Read the model definition and answer for the solid it produces. Units are mm, in the model's axes. A direction names the side the tool comes from. Round coordinates to 2 decimals unless told otherwise and drop trailing zeros. Loops run counter-clockwise (first coordinate to the right, second up) from the corner with the lowest first, then second, coordinate; pieces in that order, holes last. Notation, with made-up numbers: (23.5, 23.5) - (42.5, 23.5) arc R27 ccw to (42.5, 44.5) - close; hole circle Ø9 at (36.5, -9). An arc over 180 degrees is marked (long way). Use one line per item in the form item = value. Start each with the question number.
```python
from build123d import *

# Parameters (mm, degrees)
SKETCH1_R           = 45
SKETCH1_R_2         = 25
BOSS_EXTRUDE1_DEPTH = 15
CUT_EXTRUDE1_START  = -3
SKETCH2_R           = 45
SKETCH2_R_2         = 40
CUT_EXTRUDE1_DEPTH  = 3
SKETCH3_R           = 2
CUT_EXTRUDE2_DEPTH  = 11
CHAMFER1_SIZE       = 1


with BuildPart() as part:
    # Sketch1 → Boss-Extrude1 (new body)
    with BuildSketch(Plane.XY):
        Circle(SKETCH1_R)
        Circle(SKETCH1_R_2, mode=Mode.SUBTRACT)
    extrude(amount=BOSS_EXTRUDE1_DEPTH)

    # Sketch2 → Cut-Extrude1 (cut)
    with BuildSketch(Plane.XY.offset(15).offset(CUT_EXTRUDE1_START)):
        Circle(SKETCH2_R)
        Circle(SKETCH2_R_2, mode=Mode.SUBTRACT)
    extrude(amount=CUT_EXTRUDE1_DEPTH, mode=Mode.SUBTRACT)

    # Sketch3 → Cut-Extrude2 (cut)
    with BuildSketch(Plane(origin=(0, 0, 0), x_dir=(-1, 0, 0), z_dir=(0, 0, -1))):
        with Locations((0, 36.5)):
            Circle(SKETCH3_R)
        with Locations((31.609927238, 18.25)):
            Circle(SKETCH3_R)
        with Locations((31.609927238, -18.25)):
            Circle(SKETCH3_R)
        with Locations((0, -36.5)):
            Circle(SKETCH3_R)
        with Locations((-31.609927238, -18.25)):
            Circle(SKETCH3_R)
        with Locations((-31.609927238, 18.25)):
            Circle(SKETCH3_R)
    extrude(amount=-CUT_EXTRUDE2_DEPTH, mode=Mode.SUBTRACT)

    # Chamfer1
    chamfer1_edges = [part.edges().sort_by_distance(p)[0] for p in [
        (-40, 0, 15),
        (-25, 0, 0),
    ]]
    chamfer(chamfer1_edges, length=CHAMFER1_SIZE)


solid = part.part
```
1) A cutting plane is placed at B-B on z = 6.75. Write down the section's boundary in (x, y), plus the area to 3 significant figures.
2) For faces 5 (the flat face through (-0.5, -25.5, 15)), 6 (the flat face through (32, -18, 11)), 7 (the cylindrical face through (-8.67, -39.05, 12.99)), determine the directions among +Z, -Z, +X, -X, +Y, -Y from which every point of the face is accessible in a straight line to the end or side of a thin tool.
3) A cutting plane is placed at A-A on y = 0. Write down the section's boundary in (x, z).
4) Determine the mould class of faces 1 (the flat face through (-30.2, -26.5, 12)), 2 (the flat face through (-32, 18, 11)), 3 (the cylindrical face through (30.535, -16.564, 5.423)), 4 (the cylindrical face through (20.765, -39.923, 5.916)) for opening direction X: +X half, -X half, draft (parallel to the pull), parting line (faces both ways), or undercut.
5) Straight lines are drawn through the part: line 1 (Y direction, x = 0, z = 8.75); line 2 (X direction, y = -0.5, z = 10.25) (3 decimals); line 3 (Y direction, x = 7.5, z = 11). For each, find the intervals that lie inside material, in ascending order. Write a range as from..to.
6) Flat-ended cylindrical pins translate along their axes: pin 1 (3 mm diameter, centred on x = 0.5, y = 36, fed in from -Z); pin 2 (2 mm diameter, centred on x = 31.5, y = -18, fed in from -Z); pin 3 (3 mm diameter, centred on x = 16.5, z = 3, fed in from +Y); pin 4 (6 mm diameter, centred on x = -15, z = 6.5, fed in from -Y). Find the tip coordinate at first contact, or state that the pin passes through.
Checks:
q1.outline = circle Ø90 at (0, 0); hole circle Ø4 at (-31.61, -18.25); hole circle Ø4 at (-31.61, 18.25); hole circle Ø50 at (0, 0); hole circle Ø4 at (0, -36.5); hole circle Ø4 at (0, 36.5); hole circle Ø4 at (31.61, -18.25); hole circle Ø4 at (31.61, 18.25)
q1.area = 4,320 mm²
q2.face_5 = +Z, +X, -X, +Y, -Y
q2.face_6 = -Z
q2.face_7 = +Z
q3.outline = (-45, 0) - (-26, 0) - (-25, 1) - (-25, 15) - (-39, 15) - (-40, 14) - (-40, 12) - (-45, 12) - close; (25, 1) - (26, 0) - (45, 0) - (45, 12) - (40, 12) - (40, 14) - (39, 15) - (25, 15) - close
q4.face_1 = draft
q4.face_2 = undercut
q4.face_3 = undercut
q4.face_4 = parting line
q5.line_1 = -45..-38.5, -34.5..-25, 25..34.5, 38.5..45
q5.line_2 = -44.997..-24.995, 24.995..44.997
q5.line_3 = -44.37..-23.85, 23.85..44.37
q6.pin_1 = 0
q6.pin_2 = 11
q6.pin_3 = 42.43
q6.pin_4 = -43.37
